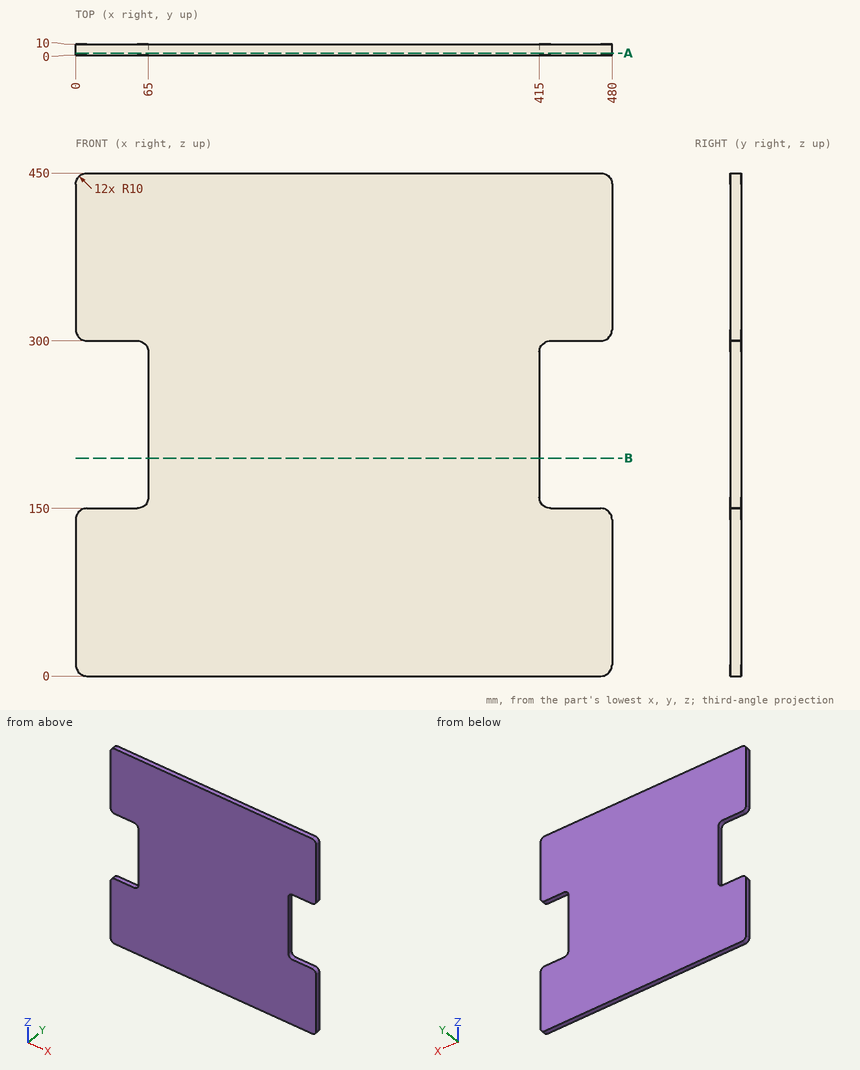
Input: dimensioned drawing with shaded views. Units: mm. Origin: part minimum x, y, z. Coordinates: 2 decimals unless noted, no trailing zeros. Write each loop counter-clockwise with the first axis right and the second up, starting at its lowest first coordinate (ties: lowest second). Pieces come first, ordered by that corner, then holes. Notation, with made-up numbers: M 69,47 L 94,47 A22 cw 94,62 Z; hole C 82.25,-38 d3. An arc over 180 degrees is marked long. Use one line per item in the form item = value.
Q1. Section A-A (y = 1.75). Return loops of the section in (x, z), plus the area to 3 significant figures.
Answer below:
outline = M 0,10 A10 ccw 10,0 L 470,0 A10 ccw 480,10 L 480,140 A10 ccw 470,150 L 425,150 A10 cw 415,160 L 415,290 A10 cw 425,300 L 470,300 A10 ccw 480,310 L 480,440 A10 ccw 470,450 L 10,450 A10 ccw 0,440 L 0,310 A10 ccw 10,300 L 55,300 A10 cw 65,290 L 65,160 A10 cw 55,150 L 10,150 A10 ccw 0,140 Z
area = 196,000 mm²
Q2. Section B-B (z = 195). Return loops of the section in (x, y).
Answer below:
outline = M 65,0 L 415,0 L 415,10 L 65,10 Z
Q3. Material intervals for probe 1 along Z at (x, y) = (448, 4); probe 2 along X at (y, z) = (7.5, 243.5); probe 3 along X at (y, z) = (4, 145), sorted ascending. Write a range as from..to.
Answer below:
probe_1 = 0..150, 300..450
probe_2 = 65..415
probe_3 = 1.34..478.66
